Can you work these out from the model? Positions are in its coordinate system, mm. Face numbers are marked on the shaded views. A direction names the side the tool comes from. Give positions to 0.01 mm unless a question says otherwise; leave off trailing zeros. Order: outer loops, then holes, each group sorted by start corner. A loop starts at its lowest first (then second) coordinate and runs counter-clockwise, first axis right, second up. Notation, with made-up numbers: (-11.75, 31) - (8.25, 31) arc R18 cw to (8.25, 62) - close; hole circle Ø11 at (-3, 11.5). An arc over 180 degrees is marked (long way). Return JSON: item names as keys, results as strings.
```python
from build123d import *

# Parameters (mm, degrees)
SKETCH_1_W                = 25
SKETCH_1_H                = 60
EXTRUDE_1_DEPTH           = 10
SKETCH_2_R                = 7.6
CUT_EXTRUDE_1_DEPTH       = 20
SKETCH_3_W                = 25
SKETCH_3_H                = 10
EXTRUDE_2_DEPTH           = 20
CHAMFER_1_SIZE            = 2
HOLE_WIZARD_1_D           = 4.5
HOLE_WIZARD_1_DEPTH       = 15
HOLE_WIZARD_1_CBORE_D     = 8
HOLE_WIZARD_1_CBORE_DEPTH = 4.6
HOLE_WIZARD_1_TIP         = 1.351936393
MM_1_D                    = 4
MM_1_DEPTH                = 15
MM_1_TIP                  = 1.201721238
HOLE_WIZARD_M3_1_D        = 2.5
HOLE_WIZARD_M3_1_DEPTH    = 15
HOLE_WIZARD_M3_1_TIP      = 0.751075774


with BuildPart() as part:
    # 草图1 → 凸台-拉伸1 (new body)
    with BuildSketch(Plane(origin=(0, 0, 0), x_dir=(1, 0, 0), z_dir=(0, 1, 0))):
        Rectangle(SKETCH_1_W, SKETCH_1_H)
    extrude(amount=EXTRUDE_1_DEPTH)

    # 草图2 → 切除-拉伸1 (cut)
    with BuildSketch(Plane.XZ):
        with Locations(Location((0, -14, 0), (0, 0, 270))):
            Circle(SKETCH_2_R)
    extrude(amount=-CUT_EXTRUDE_1_DEPTH, mode=Mode.SUBTRACT)

    # 草图3 → 凸台-拉伸2 (add)
    with BuildSketch(Plane(origin=(0, 10, 0), x_dir=(1, 0, 0), z_dir=(0, 1, 0))):
        with Locations((0, -25)):
            Rectangle(SKETCH_3_W, SKETCH_3_H)
    extrude(amount=EXTRUDE_2_DEPTH)

    # 倒角1
    chamfer_1_edges = [part.edges().sort_by_distance(p)[0] for p in [
        (-12.5, 30, 25),
        (12.5, 30, 25),
        (-12.5, 5, -30),
        (12.5, 5, -30),
    ]]
    chamfer(chamfer_1_edges, length=CHAMFER_1_SIZE)

    # 打孔尺寸(%根据)内六角圆柱头螺钉的类型1
    with Locations(Plane(origin=(0, 0, 20), x_dir=(-1, 0, 0), z_dir=(0, 0, -1))):
        with Locations((7, 20), (-7, 20)):
            CounterBoreHole(HOLE_WIZARD_1_D / 2, HOLE_WIZARD_1_CBORE_D / 2, HOLE_WIZARD_1_CBORE_DEPTH, depth=HOLE_WIZARD_1_DEPTH)
            with Locations((0, 0, -(HOLE_WIZARD_1_DEPTH + HOLE_WIZARD_1_TIP / 2))):  # 118° drill point
                Cone(0, HOLE_WIZARD_1_D / 2, HOLE_WIZARD_1_TIP, mode=Mode.SUBTRACT)

    # 大小mm 暗销孔1
    with Locations(Plane(origin=(0, 0, 20), x_dir=(-1, 0, 0), z_dir=(0, 0, -1))):
        with Locations((0, 26.5), (0, 14)):
            Hole(MM_1_D / 2, depth=MM_1_DEPTH)
            with Locations((0, 0, -(MM_1_DEPTH + MM_1_TIP / 2))):  # 118° drill point
                Cone(0, MM_1_D / 2, MM_1_TIP, mode=Mode.SUBTRACT)

    # M3 螺纹孔1
    with Locations(Plane(origin=(0, 0, 0), x_dir=(-1, 0, 0), z_dir=(0, -1, 0))):
        with Locations((0, 26), (0, 2)):
            Hole(HOLE_WIZARD_M3_1_D / 2, depth=HOLE_WIZARD_M3_1_DEPTH)
            with Locations((0, 0, -(HOLE_WIZARD_M3_1_DEPTH + HOLE_WIZARD_M3_1_TIP / 2))):  # 118° drill point
                Cone(0, HOLE_WIZARD_M3_1_D / 2, HOLE_WIZARD_M3_1_TIP, mode=Mode.SUBTRACT)


solid = part.part
```
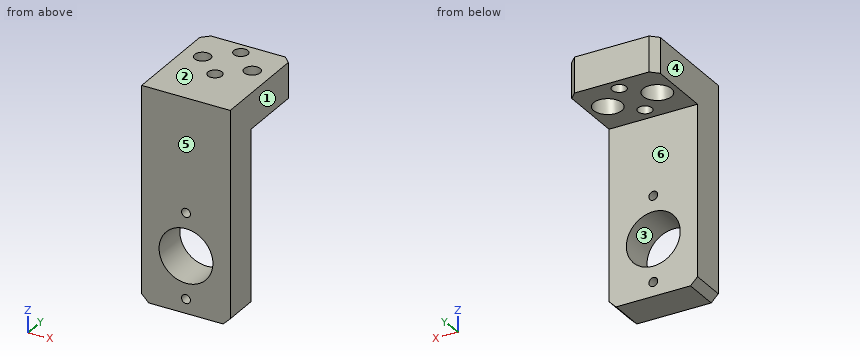
1. Suppose I cut it at A-A (y = 14). List the corners of the cut face in (x, z) for me, plus the area to 3 significant figures.
Checks:
{"outline": "(-12.5, 20) - (-2, 20) - (-2, 30) - (-12.5, 30) - close; (2, 20) - (12.5, 20) - (12.5, 30) - (2, 30) - close", "area": "210 mm^2"}
2. Suppose I cut it at D-D (y = 20). List the corners of the cut face in (x, z) for me.
Checks:
{"outline": "(-12.5, 20) - (-11, 20) - (-11, 24.6) - (-9.25, 24.6) - (-9.25, 30) - (-12.5, 30) - close; (-4.75, 24.6) - (-3, 24.6) - (-3, 20) - (3, 20) - (3, 24.6) - (4.75, 24.6) - (4.75, 30) - (-4.75, 30) - close; (9.25, 24.6) - (11, 24.6) - (11, 20) - (12.5, 20) - (12.5, 30) - (9.25, 30) - close"}
3. Thinking about a two-plate mould opening in X: for the marked faces 1, 2, 3 and 4, which applies, +X half, -X half, draft (parallel to the pull), parting line (faces both ways), or undercut?
Checks:
{"face 1": "+X half", "face 2": "draft", "face 3": "undercut", "face 4": "-X half"}
4. On a 3-axis mill with a long thin cutter (end or side, diameter ignored), from which of +Z, -Z, +X, -X, +Y, -Y can I reach the whole of each face in a straight line? I mean the marked faces 5 and 6. Say none if no direction works.
Checks:
{"face 5": "+Z, -Z, +X, -X, -Y", "face 6": "-Z, +X, -X, +Y"}
5. If I drill on L1, parallel to Z at x = -0.5, y = 7.75; L2, parallel to Y at x = 1.75, z = 25; L3, parallel to X at y = 4.25, z = -14, over which ranges is the centre line in solid material (lowest first)? Write a range as [from, to].
Checks:
{"L1": "[-30, -27.15], [-24.85, -21.58], [-6.42, -3.15], [-0.85, 30]", "L2": "[0, 13.03], [14.97, 25.53], [27.47, 30]", "L3": "[-12.5, -7.6], [7.6, 12.5]"}
6. Suppose I cut it at B-B (x = 0). List the corners of the cut face in (y, z) for me.
Checks:
{"outline": "(0, -30) - (10, -30) - (10, -27.25) - (0, -27.25) - close; (0, -24.75) - (10, -24.75) - (10, -21.6) - (0, -21.6) - close; (0, -6.4) - (10, -6.4) - (10, -3.25) - (0, -3.25) - close; (0, -0.75) - (10, -0.75) - (10, 20) - (12, 20) - (12, 30) - (0, 30) - close; (16, 20) - (24.5, 20) - (24.5, 30) - (16, 30) - close; (28.5, 20) - (30, 20) - (30, 30) - (28.5, 30) - close"}
7. For pin 1 Ø1.5 at (x, z) = (0, -26) entering from +Y; pin 2 Ø4 at (x, y) = (7.5, 20) entering from -Z; pin 3 Ø1 at (x, y) = (-2.5, 13.5) entering from -Z; pin 4 Ø8 at (x, z) = (-1, 8.5) entering from +Y, each with a flat end and sliding along its axis, tell me the tip position at first contact or that it passes through.
Checks:
{"pin 1": "through", "pin 2": "z = 24.6", "pin 3": "z = 20", "pin 4": "y = 10"}
8. Suppose I cut it at C-C (z = -2). List the corners of the cut face in (x, y) for me, plus the area to 3 significant figures.
Checks:
{"outline": "(-12.5, 0) - (-1.25, 0) - (-1.25, 10) - (-12.5, 10) - close; (1.25, 0) - (12.5, 0) - (12.5, 10) - (1.25, 10) - close", "area": "225 mm^2"}
